The figure shows three views and two pictorial views of one solid part (mm, origin at its lowest corner). Answer the questions. A direction names the side the tool comes from. Coordinates: 2 decimals unless noted, no trailing zeros. Loops run counter-clockwise (first coordinate to the right, second up) from the corner with the lowest first, then second, coordinate; pieces in that order, holes last. Notation, with made-up numbers: (37, 36) -> (85, 36) arc R10 ccw to (85, 43) -> close; hole circle Ø11 at (-38.5, 54.25). An arc over 180 degrees is marked (long way). Answer as a JSON object with one key per item and string values. Group by question number.
1) Which of the six approach directions +Z, -Z, +X, -X, +Y, -Y give full straight-line access (tool end or side, diameter ignored) to the marked faces 1 and 2?
2) Consider probe 1 along Z at (x, y) = (14, 7.75); probe 2 along Z at (x, y) = (14.5, 2.5); probe 3 along X at (y, z) = (15.5, 27) (3 decimals). Determine where each line is inside the solid, lowest interval first. Write a range as [from, to].
3) Determine the mould class of the marked faces 3, 4 and 5 for opening direction Z: released by +Z, released by -Z, zero draft, split by the parting line, or undercut.
4) Section A-A, the plane x = 20 is taken. Give the vertices of the cut face in (y, z), plus the area to 3 significant figures.
5) Section B-B, the plane z = 20 is taken. Give the vertices of the cut face in (x, y), plus the area to 3 significant figures.
6) Flat-ended cylindrical pins translate along their axes: P1, Ø4, axis at x = 33.5, y = 17, coming from the +Z side; P2, Ø22, axis at x = 20, z = 20, coming from the -Y side; P3, Ø8, axis at x = 31.5, z = 16.5, coming from the -Y side; P4, Ø5, axis at y = 10.5, z = 11.5, coming from the +X side. Find the tip coordinate at first contact, or state that the pin passes through.
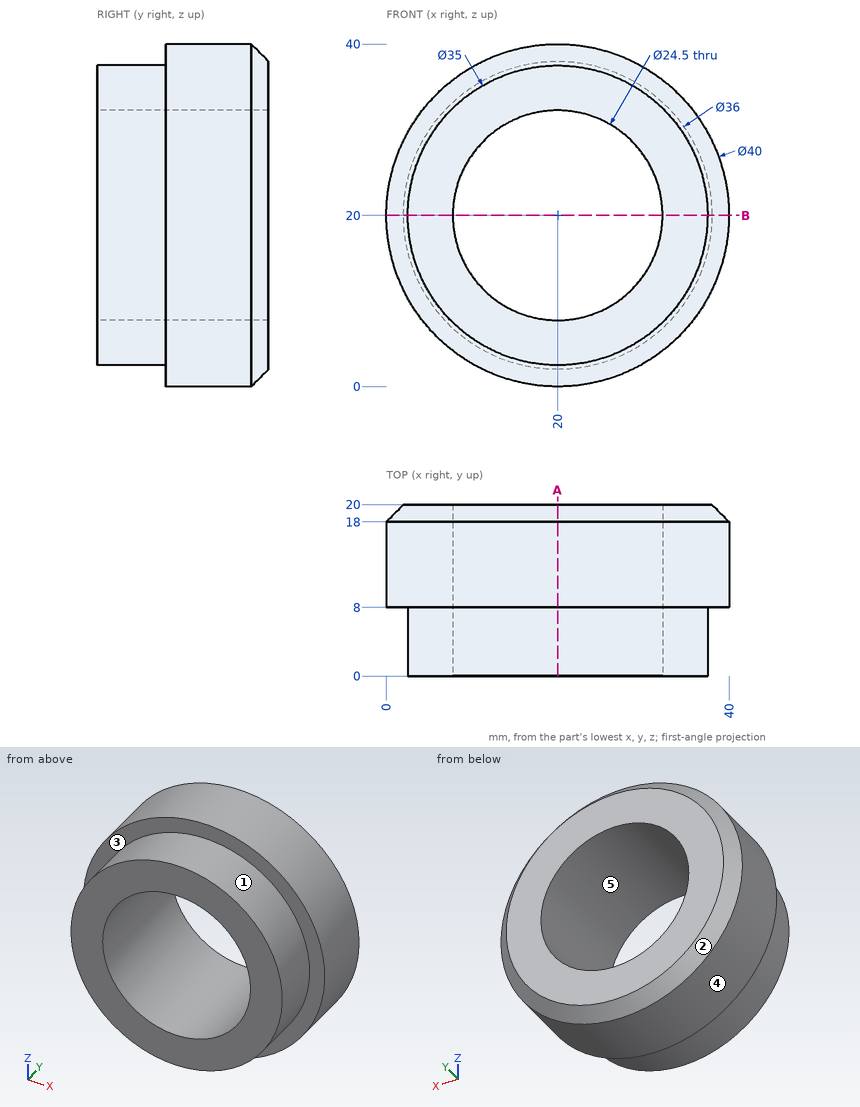
Determined:
{
 "1": {"face 1": "-Y", "face 2": "+Y"},
 "2": {"probe 1": "[3.56, 9.32], [30.68, 36.44]", "probe 2": "[3.39, 9.05], [30.95, 36.61]", "probe 3": "[1.265, 9.947], [30.053, 38.735]"},
 "3": {"face 3": "zero draft", "face 4": "split by the parting line", "face 5": "undercut"},
 "4": {"outline": "(0, 2.5) -> (8, 2.5) -> (8, 0) -> (18, 0) -> (20, 2) -> (20, 7.75) -> (0, 7.75) -> close; (0, 32.25) -> (20, 32.25) -> (20, 38) -> (18, 40) -> (8, 40) -> (8, 37.5) -> (0, 37.5) -> close", "area": "266 mm²"},
 "5": {"outline": "(0, 8) -> (2.5, 8) -> (2.5, 0) -> (7.75, 0) -> (7.75, 20) -> (2, 20) -> (0, 18) -> close; (32.25, 0) -> (37.5, 0) -> (37.5, 8) -> (40, 8) -> (40, 18) -> (38, 20) -> (32.25, 20) -> close", "area": "266 mm²"},
 "6": {"P1": "z = 36.36", "P2": "through", "P3": "y = 0", "P4": "x = 39.08"}
}
